Build history of the part. All positions in model axes, mm. Give positions to 0.01 mm unless a question says otherwise; leave off trailing zeros. Order: outer loops, then holes, each group sorted by start corner. A loop starts at its lowest first (then second) coordinate and runs counter-clockwise, first axis right, second up. Notation, with made-up numbers: (69, 53) -> (77, 53) arc R9 ccw to (77, 66) -> close; hole circle Ø11 at (67, 25). An arc over 180 degrees is marked (long way). Use a Markdown table: item, result. Add a question column.
```python
from build123d import *

# Parameters (mm, degrees)
SKETCH1_R           = 15
BOSS_EXTRUDE1_DEPTH = 15
CHAMFER1_SIZE       = 1


with BuildPart() as part:
    # Sketch1 → Boss-Extrude1 (new body)
    with BuildSketch(Plane.XY):
        Polygon((22.078741188, -11.727283895), (21.195496365, 13.257108805), (-0.883244823, 24.9843927), (-22.078741188, 11.727283895), (-21.195496365, -13.257108805), (0.883244823, -24.9843927), align=None)
        Circle(SKETCH1_R, mode=Mode.SUBTRACT)
    extrude(amount=BOSS_EXTRUDE1_DEPTH)

    # Chamfer1
    chamfer1_edges = [part.edges().sort_by_distance(p)[0] for p in [
        (-15, 0, 0),
        (-15, 0, 15),
    ]]
    chamfer(chamfer1_edges, length=CHAMFER1_SIZE)


solid = part.part
```
(1) Band-saw the part on D-D on y = -18.5. Give the cut face in (x, z), plus the area to 3 significant figures.
(2) Pin check, flat tips, straight feed: pin 1 Ø4 at (x, z) = (-9.5, 12) entering from +Y; pin 2 Ø1 at (x, z) = (-0.5, 11) entering from +Y; pin 3 Ø3 at (x, z) = (2.5, 9) entering from +Y; pin 4 Ø8 at (x, z) = (16, 2) entering from +Y. Stop position of each tip, or through.
(3) Wall check: probe 1 along X at (y, z) = (-8, 8); probe 2 along Y at (x, z) = (-7, 9.75); probe 3 along X at (y, z) = (9.5, 9.5). Give the ranges that are in metal, low to high.
(4) Band-saw the part on A-A on z = 10.5. Give the cut face in (x, y), plus the area to 3 significant figures.
(5) Band-saw the part on B-B on y = 0. Give the cut face in (x, z), plus the area to 3 significant figures.
(6) Mould opens along X. For faces 1 (the face through (-14.985, 0.66, 7.409)), 2 (the face through (-10.31, -19.04, 7.4)), 3 (the face through (-0.3, -16.3, 0)) say: released by +X, released by -X, zero draft, split by the parting line, or undercut.
(7) Band-saw the part on C-C on x = 0. Give the cut face in (y, z), plus the area to 3 significant figures.
Response:
| question | item | result |
|---|---|---|
| 1 | outline | (-11.32, 0) -> (11.25, 0) -> (11.25, 15) -> (-11.32, 15) -> close |
| 1 | area | 339 mm² |
| 2 | pin 1 | stops at y = 20.85 |
| 2 | pin 2 | stops at y = 24.98 |
| 2 | pin 3 | stops at y = 23.98 |
| 2 | pin 4 | stops at y = 18.14 |
| 3 | probe 1 | x = -21.38 to -12.69, 12.69 to 21.95 |
| 3 | probe 2 | y = -20.8 to -13.27, 13.27 to 21.16 |
| 3 | probe 3 | x = -22 to -11.61, 11.61 to 21.33 |
| 4 | outline | (-22.08, 11.73) -> (-21.2, -13.26) -> (0.88, -24.98) -> (22.08, -11.73) -> (21.2, 13.26) -> (-0.88, 24.98) -> close; hole circle Ø30 at (0, 0) |
| 4 | area | 917 mm² |
| 5 | outline | (-21.66, 0) -> (-16, 0) -> (-15, 1) -> (-15, 14) -> (-16, 15) -> (-21.66, 15) -> close; (15, 1) -> (16, 0) -> (21.66, 0) -> (21.66, 15) -> (16, 15) -> (15, 14) -> close |
| 5 | area | 198 mm² |
| 6 | face 1 | undercut |
| 6 | face 2 | released by -X |
| 6 | face 3 | zero draft |
| 7 | outline | (-24.52, 0) -> (-16, 0) -> (-15, 1) -> (-15, 14) -> (-16, 15) -> (-24.52, 15) -> close; (15, 1) -> (16, 0) -> (24.52, 0) -> (24.52, 15) -> (16, 15) -> (15, 14) -> close |
| 7 | area | 283 mm² |
